Part model, mm, in its own coordinate system. A direction names the side the tool comes from. Coordinates: 2 decimals unless noted, no trailing zeros. Order: outer loops, then holes, each group sorted by start corner. A loop starts at its lowest first (then second) coordinate and runs counter-clockwise, first axis right, second up.
1) Cut at A-A (y = 0). List the corners of the cut face in (x, z).
2) Tool access for faces 3 (the cylindrical face through (-1.46, 6.59, 0.25)), 4 (the cylindrical face through (-4.282, -4.203, 0.746)), 5 (the cylindrical face through (-1.46, -6.59, 1.25)): list every direction of +Z, -Z, +X, -X, +Y, -Y with a clear straight run to the whole face (end or side of a thin tool).
3) Wall check: L1, parallel to Y at x = 0, z = 1.1; L2, parallel to Y at x = 0, z = 0.75; L3, parallel to X at y = 0.25, z = 1.25. Give the ranges that are in metal, low to high.
4) Cut at C-C (y = -3). List the corners of the cut face in (x, z).
5) Mould opens along Y. For faces 1 (the flat face through (1.4, -1.4, 0.5)), 2 (the cylindrical face through (6.466, 2.681, 0.74)) say: +Y half, -Y half, draft (parallel to the pull), parting line (faces both ways), or undercut.
6) Cut at D-D (x = -5.5). List the corners of the cut face in (y, z), and give its area (3 significant figures).
7) Pin check, flat tips, straight feed: pin 1 Ø0.6 at (y, z) = (-4, 0.5) entering from -X; pin 2 Ø0.6 at (y, z) = (5, 1) entering from +X; pin 3 Ø1.5 at (x, y) = (3, -2) entering from +Z. Stop position of each tip, or through.
```python
from build123d import *
from build123d.topology import SkipClean

# Parameters (mm, degrees)
HUB_CORE_SKETCH_R           = 2.25
HUB_CORE_DEPTH              = 0.5
HUB_FLANGE_SKETCH_R         = 6
HUB_FLANGE_6_DEPTH          = 0.5
FRONT_HUB_BOSS_SKETCH_R     = 2.25
FRONT_HUB_BOSS_DEPTH        = 0.5
CROSS_START                 = -0.5
CROSS_SLOT_CUT_DEPTH        = 0.5
WEB_START                   = -0.5
WEB_RING_SKETCH_R           = 6.75
WEB_RING_SKETCH_R_2         = 6
WEB_RING_13_5_DEPTH         = 0.5
FRONT_START                 = -0.5
FRONT_HUB_HOLE_SKETCH_R     = 2.25
FRONT_HUB_HOLE_CUT_DEPTH    = 0.5
BACK_HUB_RECESS_SKETCH_R    = 2.25
BACK_HUB_RECESS_CUT_DEPTH   = 0.5
HUB_RING_A_SKETCH_R         = 1.5
HUB_RING_A_DEPTH            = 0.5
HUB_START                   = 0.5
HUB_RING_B_SKETCH_R         = 1.5
HUB_RING_B_DEPTH            = 0.5
SPOKE_1_DEPTH               = 1.5
SPOKE_1_GROOVE_A_DEPTH      = 0.625
SPOKE_1_GROOVE_B_DEPTH      = 0.625
SPOKE_2_DEPTH               = 1.5
SPOKE_3_DEPTH               = 1.5
SPOKE_4_DEPTH               = 1.5
SPOKE_GROOVES_A_DEPTH       = 0.65
SPOKE_GROOVES_B_DEPTH       = 0.65
CROSS_SPOKES_DEPTH          = 1.5
CROSS_SPOKES_2_DEPTH        = 1.5
CROSS_SPOKES_3_DEPTH        = 1.5
CROSS_SPOKES_4_DEPTH        = 1.5
CROSS_SPOKE_GROOVES_A_DEPTH = 0.625
CROSS_SPOKE_GROOVES_B_DEPTH = 0.625
CENTRE_HOLE_SKETCH_R        = 1
CENTRE_HOLE_CUT_DEPTH       = 10
RIM_START                   = -0.5
RIM_RING_1_SKETCH_R         = 7
RIM_RING_1_SKETCH_R_2       = 6.75
RIM_RING_1_14_DEPTH         = 0.5
RIM_RING_2_SKETCH_R         = 7
RIM_RING_2_SKETCH_R_2       = 6.75
RIM_RING_2_14_DEPTH         = 0.5
RIM_START_2                 = 0.5
RIM_RING_3_SKETCH_R         = 7
RIM_RING_3_SKETCH_R_2       = 6.75
RIM_RING_3_14_DEPTH         = 0.5


with BuildPart() as part:
    # Hub Core Sketch → Hub Core (new body)
    with BuildSketch(Plane.XY):
        Circle(HUB_CORE_SKETCH_R)
    extrude(amount=HUB_CORE_DEPTH)

    # Hub Flange Sketch → Hub Flange Ø6 (add)
    with BuildSketch(Plane.XY.offset(0.5)):
        Circle(HUB_FLANGE_SKETCH_R)
    extrude(amount=HUB_FLANGE_6_DEPTH)

    # Front Hub Boss Sketch → Front Hub Boss (add)
    with BuildSketch(Plane.XY.offset(1)):
        Circle(FRONT_HUB_BOSS_SKETCH_R)
    extrude(amount=FRONT_HUB_BOSS_DEPTH)

    # Cross Slot Sketch → Cross Slot Cut (cut)
    with SkipClean():  # the faces are left unmerged after this step: merging them gives an invalid solid
        with BuildSketch(Plane.XY.offset(1).offset(CROSS_START)):
            with BuildLine():
                ThreePointArc((-2.121320344, 0.75), (-1.590990258, 1.590990258), (-0.75, 2.121320344))
                Line((-0.75, 2.121320344), (-0.75, 5.95294045))
                ThreePointArc((-0.75, 5.95294045), (-4.242640687, 4.242640687), (-5.95294045, 0.75))
                Line((-5.95294045, 0.75), (-2.121320344, 0.75))
            make_face()
            with BuildLine():
                Line((0.75, 5.95294045), (0.75, 2.121320344))
                ThreePointArc((0.75, 2.121320344), (1.590990258, 1.590990258), (2.121320344, 0.75))
                Line((2.121320344, 0.75), (5.95294045, 0.75))
                ThreePointArc((5.95294045, 0.75), (4.242640687, 4.242640687), (0.75, 5.95294045))
            make_face()
            with BuildLine():
                ThreePointArc((2.121320344, -0.75), (1.590990258, -1.590990258), (0.75, -2.121320344))
                Line((0.75, -2.121320344), (0.75, -5.95294045))
                ThreePointArc((0.75, -5.95294045), (4.242640687, -4.242640687), (5.95294045, -0.75))
                Line((5.95294045, -0.75), (2.121320344, -0.75))
            make_face()
            with BuildLine():
                Line((-0.75, -5.95294045), (-0.75, -2.121320344))
                ThreePointArc((-0.75, -2.121320344), (-1.590990258, -1.590990258), (-2.121320344, -0.75))
                Line((-2.121320344, -0.75), (-5.95294045, -0.75))
                ThreePointArc((-5.95294045, -0.75), (-4.242640687, -4.242640687), (-0.75, -5.95294045))
            make_face()
        extrude(amount=CROSS_SLOT_CUT_DEPTH, mode=Mode.SUBTRACT)

    # Web Ring Sketch → Web Ring Ø13.5 (add)
    with SkipClean():  # the faces are left unmerged after this step: merging them gives an invalid solid
        with BuildSketch(Plane.XY.offset(1).offset(WEB_START)):
            Circle(WEB_RING_SKETCH_R)
            Circle(WEB_RING_SKETCH_R_2, mode=Mode.SUBTRACT)
        extrude(amount=WEB_RING_13_5_DEPTH)

    # Front Hub Hole Sketch → Front Hub Hole Cut (cut)
    with SkipClean():  # the faces are left unmerged after this step: merging them gives an invalid solid
        with BuildSketch(Plane.XY.offset(1.5).offset(FRONT_START)):
            with Locations(Location((0, 0, 0), (0, 0, 199.471220634))):
                Circle(FRONT_HUB_HOLE_SKETCH_R)
        extrude(amount=FRONT_HUB_HOLE_CUT_DEPTH, mode=Mode.SUBTRACT)

    # Back Hub Recess Sketch → Back Hub Recess Cut (cut)
    with BuildSketch(Plane(origin=(0, 0, 0), x_dir=(-1, 0, 0), z_dir=(0, 0, -1))):
        Circle(BACK_HUB_RECESS_SKETCH_R)
    extrude(amount=-BACK_HUB_RECESS_CUT_DEPTH, mode=Mode.SUBTRACT)

    # Hub Ring A Sketch → Hub Ring A (add)
    with BuildSketch(Plane(origin=(0, 0, 0.5), x_dir=(-1, 0, 0), z_dir=(0, 0, -1))):
        Circle(HUB_RING_A_SKETCH_R)
    extrude(amount=HUB_RING_A_DEPTH)

    # Hub Ring B Sketch → Hub Ring B (add)
    with BuildSketch(Plane.XY.offset(1).offset(HUB_START)):
        with Locations(Location((0, 0, 0), (0, 0, 180))):
            Circle(HUB_RING_B_SKETCH_R)
    extrude(amount=-HUB_RING_B_DEPTH)

    # Centre Hole Sketch → Centre Hole Cut (cut)
    with BuildSketch(Plane.XY.offset(1.5)):
        Circle(CENTRE_HOLE_SKETCH_R)
    extrude(amount=-CENTRE_HOLE_CUT_DEPTH, mode=Mode.SUBTRACT)

    # Rim Ring 1 Sketch → Rim Ring 1 Ø14 (add)
    with BuildSketch(Plane.XY.offset(1).offset(RIM_START)):
        Circle(RIM_RING_1_SKETCH_R)
        Circle(RIM_RING_1_SKETCH_R_2, mode=Mode.SUBTRACT)
    extrude(amount=RIM_RING_1_14_DEPTH)

    # Rim Ring 2 Sketch → Rim Ring 2 Ø14 (add)
    with BuildSketch(Plane.XY.offset(1)):
        Circle(RIM_RING_2_SKETCH_R)
        Circle(RIM_RING_2_SKETCH_R_2, mode=Mode.SUBTRACT)
    extrude(amount=RIM_RING_2_14_DEPTH)

    # Rim Ring 3 Sketch → Rim Ring 3 Ø14 (add)
    with BuildSketch(Plane(origin=(0, 0, 0.5), x_dir=(-1, 0, 0), z_dir=(0, 0, -1)).offset(RIM_START_2)):
        with Locations(Location((0, 0, 0), (0, 0, 180))):
            Circle(RIM_RING_3_SKETCH_R)
        with Locations(Location((0, 0, 0), (0, 0, 180))):
            Circle(RIM_RING_3_SKETCH_R_2, mode=Mode.SUBTRACT)
    extrude(amount=-RIM_RING_3_14_DEPTH)


with BuildPart() as body_2:
    # Spoke 1 Sketch → Spoke 1 (new body)
    with BuildSketch(Plane.XZ.offset(0.75)):
        Polygon((-1.5, 1.5), (-1.5, 1), (-6.75, 1), (-5.25, 1.5), align=None)
    extrude(amount=-SPOKE_1_DEPTH)

    # Spoke 1 Groove A Sketch → Spoke 1 Groove A (cut)
    with BuildSketch(Plane.XZ.offset(0.75)):
        Polygon((-6.75, 1), (-5.25, 1.5), (-1.5, 1.5), (-1.5, 1), align=None)
    extrude(amount=-SPOKE_1_GROOVE_A_DEPTH, mode=Mode.SUBTRACT)

    # Spoke 1 Groove B Sketch → Spoke 1 Groove B (cut)
    with BuildSketch(Plane(origin=(0, 0.75, 0), x_dir=(1, 0, 0), z_dir=(0, 1, 0))):
        Polygon((-1.5, -1.5), (-1.5, -1), (-6.75, -1), (-5.25, -1.5), align=None)
    extrude(amount=-SPOKE_1_GROOVE_B_DEPTH, mode=Mode.SUBTRACT)


with BuildPart() as body_3:
    # Spoke 2 Sketch → Spoke 2 (new body)
    with BuildSketch(Plane.XZ.offset(0.75)):
        Polygon((5.25, 1.5), (1.5, 1.5), (1.5, 1), (2.121320344, 1), (5.95294045, 1), (6.75, 1), align=None)
    extrude(amount=-SPOKE_2_DEPTH)


with BuildPart() as body_4:
    # Spoke 3 Sketch → Spoke 3 (new body)
    with BuildSketch(Plane.XZ.offset(0.75)):
        Polygon((1.5, 0), (1.5, 0.5), (6.75, 0.5), (5.25, 0), align=None)
    extrude(amount=-SPOKE_3_DEPTH)


with BuildPart() as body_5:
    # Spoke 4 Sketch → Spoke 4 (new body)
    with BuildSketch(Plane.XZ.offset(0.75)):
        Polygon((-1.5, 0), (-5.25, 0), (-6.75, 0.5), (-1.5, 0.5), align=None)
    extrude(amount=-SPOKE_4_DEPTH)


with BuildPart() as spoke_grooves_a_tool:
    # Spoke Grooves A Sketch → Spoke Grooves A (new body)
    with BuildSketch(Plane.XZ.offset(0.75)):
        Polygon((1.5, 1.5), (1.5, 1), (6.75, 1), (5.25, 1.5), align=None)
        Polygon((1.5, 0), (1.5, 0.5), (6.75, 0.5), (5.25, 0), align=None)
        Polygon((-6.75, 0.5), (-1.5, 0.5), (-1.5, 0), (-5.25, 0), align=None)
    extrude(amount=-SPOKE_GROOVES_A_DEPTH)


with BuildPart() as body_3_1:
    add(body_3.part)

    # Spoke Grooves A: cut by spoke_grooves_a_tool
    add(spoke_grooves_a_tool.part, mode=Mode.SUBTRACT)


with BuildPart() as body_4_1:
    add(body_4.part)

    # Spoke Grooves A: cut by spoke_grooves_a_tool
    add(spoke_grooves_a_tool.part, mode=Mode.SUBTRACT)


with BuildPart() as body_5_1:
    add(body_5.part)

    # Spoke Grooves A: cut by spoke_grooves_a_tool
    add(spoke_grooves_a_tool.part, mode=Mode.SUBTRACT)


with BuildPart() as spoke_grooves_b_tool:
    # Spoke Grooves B Sketch → Spoke Grooves B (new body)
    with BuildSketch(Plane(origin=(0, 0.75, 0), x_dir=(1, 0, 0), z_dir=(0, 1, 0))):
        Polygon((1.5, 0), (5.25, 0), (6.75, -0.5), (1.5, -0.5), align=None)
        Polygon((1.5, -1.5), (1.5, -1), (6.75, -1), (5.25, -1.5), align=None)
        Polygon((-6.75, -0.5), (-1.5, -0.5), (-1.5, 0), (-5.25, 0), align=None)
    extrude(amount=-SPOKE_GROOVES_B_DEPTH)


with BuildPart() as body_3_2:
    add(body_3_1.part)

    # Spoke Grooves B: cut by spoke_grooves_b_tool
    add(spoke_grooves_b_tool.part, mode=Mode.SUBTRACT)


with BuildPart() as body_4_2:
    add(body_4_1.part)

    # Spoke Grooves B: cut by spoke_grooves_b_tool
    add(spoke_grooves_b_tool.part, mode=Mode.SUBTRACT)


with BuildPart() as body_5_2:
    add(body_5_1.part)

    # Spoke Grooves B: cut by spoke_grooves_b_tool
    add(spoke_grooves_b_tool.part, mode=Mode.SUBTRACT)


with BuildPart() as body_6:
    # Cross Spokes Sketch → Cross Spokes (new body)
    with BuildSketch(Plane.ZY.offset(0.75)):
        Polygon((1, 1.5), (1, 6.75), (1.5, 5.25), (1.5, 1.5), align=None)
    extrude(amount=-CROSS_SPOKES_DEPTH)


with BuildPart() as body_7:
    # Cross Spokes Sketch → Cross Spokes 2 (new body)
    with BuildSketch(Plane.ZY.offset(0.75)):
        Polygon((0.5, 1.5), (0.5, 6.75), (0, 5.25), (0, 1.5), align=None)
    extrude(amount=-CROSS_SPOKES_2_DEPTH)


with BuildPart() as body_8:
    # Cross Spokes Sketch → Cross Spokes 3 (new body)
    with BuildSketch(Plane.ZY.offset(0.75)):
        Polygon((1, -1.5), (1, -6.75), (1.5, -5.25), (1.5, -1.5), align=None)
    extrude(amount=-CROSS_SPOKES_3_DEPTH)


with BuildPart() as body_9:
    # Cross Spokes Sketch → Cross Spokes 4 (new body)
    with BuildSketch(Plane.ZY.offset(0.75)):
        Polygon((0.5, -1.5), (0.5, -6.75), (0, -5.25), (0, -1.5), align=None)
    extrude(amount=-CROSS_SPOKES_4_DEPTH)


with BuildPart() as cross_spoke_grooves_a_tool:
    # Cross Spoke Grooves A Sketch → Cross Spoke Grooves A (new body)
    with BuildSketch(Plane.ZY.offset(0.75)):
        Polygon((1.5, 1.5), (1, 1.5), (1, 6.75), (1.5, 5.25), align=None)
        Polygon((0.5, 6.75), (0.5, 1.5), (0, 1.5), (0, 5.25), align=None)
        Polygon((1, -6.75), (1, -1.5), (1.5, -1.5), (1.5, -5.25), align=None)
        Polygon((0, -1.5), (0.5, -1.5), (0.5, -6.75), (0, -5.25), align=None)
    extrude(amount=-CROSS_SPOKE_GROOVES_A_DEPTH)


with BuildPart() as body_6_1:
    add(body_6.part)

    # Cross Spoke Grooves A: cut by cross_spoke_grooves_a_tool
    add(cross_spoke_grooves_a_tool.part, mode=Mode.SUBTRACT)


with BuildPart() as body_7_1:
    add(body_7.part)

    # Cross Spoke Grooves A: cut by cross_spoke_grooves_a_tool
    add(cross_spoke_grooves_a_tool.part, mode=Mode.SUBTRACT)


with BuildPart() as body_8_1:
    add(body_8.part)

    # Cross Spoke Grooves A: cut by cross_spoke_grooves_a_tool
    add(cross_spoke_grooves_a_tool.part, mode=Mode.SUBTRACT)


with BuildPart() as body_9_1:
    add(body_9.part)

    # Cross Spoke Grooves A: cut by cross_spoke_grooves_a_tool
    add(cross_spoke_grooves_a_tool.part, mode=Mode.SUBTRACT)


with BuildPart() as cross_spoke_grooves_b_tool:
    # Cross Spoke Grooves B Sketch → Cross Spoke Grooves B (new body)
    with BuildSketch(Plane(origin=(0.75, 0, 0), x_dir=(0, 0, -1), z_dir=(1, 0, 0))):
        Polygon((0, 1.5), (-0.5, 1.5), (-0.5, 6.75), (0, 5.25), align=None)
        Polygon((-1, 6.75), (-1, 1.5), (-1.5, 1.5), (-1.5, 5.25), align=None)
        Polygon((0, -1.5), (0, -5.25), (-0.5, -6.75), (-0.5, -1.5), align=None)
        Polygon((-1.5, -1.5), (-1.5, -5.25), (-1, -6.75), (-1, -1.5), align=None)
    extrude(amount=-CROSS_SPOKE_GROOVES_B_DEPTH)


with BuildPart() as body_6_2:
    add(body_6_1.part)

    # Cross Spoke Grooves B: cut by cross_spoke_grooves_b_tool
    add(cross_spoke_grooves_b_tool.part, mode=Mode.SUBTRACT)


with BuildPart() as body_7_2:
    add(body_7_1.part)

    # Cross Spoke Grooves B: cut by cross_spoke_grooves_b_tool
    add(cross_spoke_grooves_b_tool.part, mode=Mode.SUBTRACT)


with BuildPart() as body_8_2:
    add(body_8_1.part)

    # Cross Spoke Grooves B: cut by cross_spoke_grooves_b_tool
    add(cross_spoke_grooves_b_tool.part, mode=Mode.SUBTRACT)


with BuildPart() as body_9_2:
    add(body_9_1.part)

    # Cross Spoke Grooves B: cut by cross_spoke_grooves_b_tool
    add(cross_spoke_grooves_b_tool.part, mode=Mode.SUBTRACT)


solid = part.part
```
Geometry check:
1. outline: (-7, 0) - (-6.75, 0) - (-6.75, 0.5) - (-1.5, 0.5) - (-1.5, 0) - (-1, 0) - (-1, 1.5) - (-1.5, 1.5) - (-1.5, 1) - (-6.75, 1) - (-6.75, 1.5) - (-7, 1.5) - close; (1, 0) - (1.5, 0) - (1.5, 0.5) - (6.75, 0.5) - (6.75, 0) - (7, 0) - (7, 1.5) - (6.75, 1.5) - (6.75, 1) - (1.5, 1) - (1.5, 1.5) - (1, 1.5) - close
2. face 3: -Z
2. face 4: +Z, -Z
2. face 5: +Z
3. L1: y = -7 to -6.75, -1.5 to -1, 1 to 1.5, 6.75 to 7
3. L2: y = -7 to -1, 1 to 7
3. L3: x = -7 to -6.75, -1.48 to -0.97, 0.97 to 1.48, 6.75 to 7
4. outline: (-6.32, 0) - (-6.05, 0) - (-6.05, 0.5) - (-5.2, 0.5) - (-5.2, 1) - (-6.05, 1) - (-6.05, 1.5) - (-6.32, 1.5) - close; (-0.75, 0.5) - (0.75, 0.5) - (0.75, 1) - (-0.75, 1) - close; (5.2, 0.5) - (6.05, 0.5) - (6.05, 0) - (6.32, 0) - (6.32, 1.5) - (6.05, 1.5) - (6.05, 1) - (5.2, 1) - close
5. face 1: undercut
5. face 2: parting line
6. outline: (-4.33, 0) - (-3.91, 0) - (-3.91, 0.5) - (-2.4, 0.5) - (-2.4, 1) - (-3.91, 1) - (-3.91, 1.5) - (-4.33, 1.5) - close; (-0.75, 0.5) - (0.75, 0.5) - (0.75, 1) - (-0.75, 1) - close; (2.4, 0.5) - (3.91, 0.5) - (3.91, 0) - (4.33, 0) - (4.33, 1.5) - (3.91, 1.5) - (3.91, 1) - (2.4, 1) - close
6. area: 3.52 mm2
7. pin 1: stops at x = -5.94
7. pin 2: stops at x = 5.19
7. pin 3: passes through
